Design review of the part built by this model. Coordinates are the model's own, in mm. A direction names the side the tool comes from. Round coordinates to 2 decimals unless told otherwise and drop trailing zeros. Order: outer loops, then holes, each group sorted by start corner. A loop starts at its lowest first (then second) coordinate and runs counter-clockwise, first axis right, second up. Notation, with made-up numbers: (-8, 35) - (-3, 35) arc R19 cw to (-3, 39) - close; hole circle Ø2 at (67, 28). An arc over 180 degrees is marked (long way). Write item = value, one per line.
from build123d import *

# Parameters (mm, degrees)
SKETCH1_R           = 27
SKETCH1_R_2         = 15.5
BOSS_EXTRUDE1_DEPTH = 15


with BuildPart() as part:
    # Sketch1 → Boss-Extrude1 (new, symmetric)
    with BuildSketch(Plane.XY):
        Circle(SKETCH1_R)
        Circle(SKETCH1_R_2, mode=Mode.SUBTRACT)
    extrude(amount=BOSS_EXTRUDE1_DEPTH, both=True)

    # Sketch2 → Cut-Revolve1 (revolve, cut)
    with BuildSketch(Plane(origin=(0, 0, 0), x_dir=(1, 0, 0), z_dir=(0, 1, 0))):
        Polygon((-27, -2.5), (-27, -12.5), (-21, -10.316178594), (-21, -4.683821406), align=None)
        Polygon((-27, 2.5), (-21, 4.683821406), (-21, 10.316178594), (-27, 12.5), align=None)
    revolve(axis=Axis((0, 0, -19.218694813), (0, 0, 1)), mode=Mode.SUBTRACT)


solid = part.part
Item 1: The part is to be moulded in two halves that separate along X. For faces 1 (the face through (-2.018, 15.368, -0.21)), 2 (the face through (12, -12, -15)), 3 (the face through (-5.85, -26.36, 0.04)), say which applies: +X half, -X half, draft (parallel to the pull), parting line (faces both ways), or undercut.
Data:
face_1 = undercut
face_2 = draft
face_3 = parting line
Item 2: For line 1 along Y through (x, z) = (0, -2.25); line 2 along Y through (x, z) = (0, 8); line 3 along Z through (x, y) = (-2.5, -24), list the stretches that pass through material, from the lowest coordinate up. Write a range as [from, to].
Data:
line_1 = [-27, -15.5], [15.5, 27]
line_2 = [-21, -15.5], [15.5, 21]
line_3 = [-15, -11.46], [-3.54, 3.54], [11.46, 15]
Item 3: For faces 4 (the face through (4.634, 20.867, 4.547)), 5 (the face through (-5.85, -26.36, -13.73)), list the 3-axis set-ups (+Z, -Z, +X, -X, +Y, -Y) from which the entire face can be reached by the end or side of a thin tool; tool diameter is ignored.
Data:
face_4 = none
face_5 = +Z, -Z
Item 4: Take a section at D-D, the plane z = 5.75. State the section outline as (x, y) points.
Data:
outline = circle Ø42 at (0, 0); hole circle Ø31 at (0, 0)
Item 5: Insertion check: P1, Ø6, axis at y = -17, z = 5, coming from the +X side; P2, Ø5, axis at x = 20.5, z = -4, coming from the -Y side; P3, Ø8, axis at y = 14, z = -5, coming from the -X side. Each pin has a flat end and moves straight along its axis. Give the tip position at first contact, or say it passes through.
Data:
P1 = 22.22
P2 = -19.67
P3 = -24.71
Item 6: Take a section at C-C, the plane z = 1.25. State the section outline as (x, y) points, and give its area (3 significant figures).
Data:
outline = circle Ø54 at (0, 0); hole circle Ø31 at (0, 0)
area = 1,540 mm2
Item 7: Take a section at A-A, the plane y = 0. State the section outline as (x, z) points, and give its area (3 significant figures).
Data:
outline = (-27, -15) - (-15.5, -15) - (-15.5, 15) - (-27, 15) - (-27, 12.5) - (-21, 10.32) - (-21, 4.68) - (-27, 2.5) - (-27, -2.5) - (-21, -4.68) - (-21, -10.32) - (-27, -12.5) - close; (15.5, -15) - (27, -15) - (27, -12.5) - (21, -10.32) - (21, -4.68) - (27, -2.5) - (27, 2.5) - (21, 4.68) - (21, 10.32) - (27, 12.5) - (27, 15) - (15.5, 15) - close
area = 502 mm2
